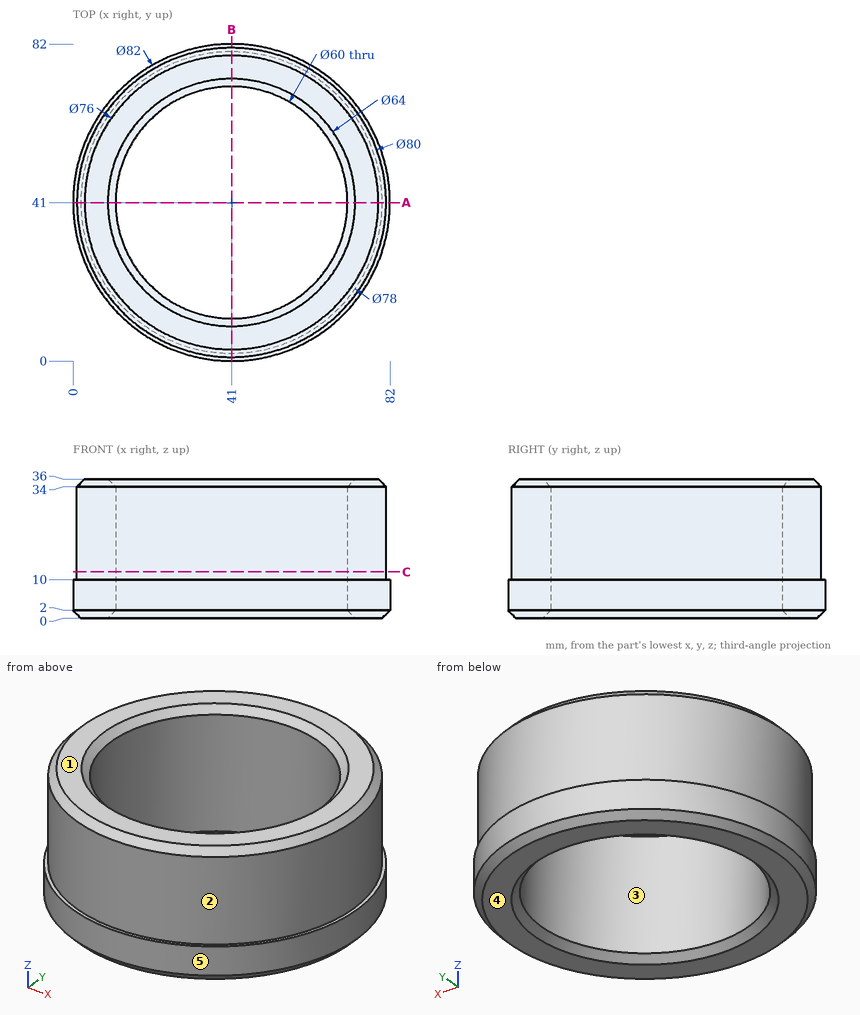
Drawing for the job (mm, zero at the part's lowest x, y, z). A direction names the side the tool comes from. Give positions to 0.01 mm unless a question says otherwise; leave off trailing zeros. Loops run counter-clockwise (first coordinate to the right, second up) from the corner with the lowest first, then second, coordinate; pieces in that order, holes last.
(1) Pin check, flat tips, straight feed: pin 1 (6 mm diameter, centred on y = 57, z = 5, fed in from -X); pin 2 (8 mm diameter, centred on x = 59, z = 20, fed in from +Y); pin 3 (1 mm diameter, centred on y = 60.5, z = 5.5, fed in from +X). Stop position of each tip, or through.
Return value:
pin 1: stops at x = 2.12
pin 2: stops at y = 78.47
pin 3: stops at x = 77.33
(2) 3-axis set-ups, long thin cutter, end or side, ignore diameter. For the marked faces 1 and 2: which of +Z, -Z, +X, -X, +Y, -Y reach the whole face in a straight line?
Return value:
face 1: +Z, +X, -X, +Y, -Y
face 2: +Z
(3) Band-saw the part on A-A (y = 41). Write the cut outline in (x, z).
Return value:
outline: (0, 2) - (2, 0) - (9, 0) - (11, 2) - (11, 34) - (9, 36) - (3, 36) - (1, 34) - (1, 10) - (0, 10) - close; (71, 2) - (73, 0) - (80, 0) - (82, 2) - (82, 10) - (81, 10) - (81, 34) - (79, 36) - (73, 36) - (71, 34) - close
(4) Band-saw the part on C-C (z = 12). Write the cut outline in (x, y), and give its area (3 significant figures).
Return value:
outline: circle Ø80 at (41, 41); hole circle Ø60 at (41, 41)
area: 2,200 mm2
(5) Drill centre lines: line 1 along Y through (x, z) = (41, 15); line 2 along X through (y, z) = (18.5, 34.5); line 3 along X through (y, z) = (38.5, 30). Where is each one in solid material? Low to high.
Return value:
line 1: y = 1 to 11, 71 to 81
line 2: x = 8.53 to 20.41, 61.59 to 73.47
line 3: x = 1.08 to 11.1, 70.9 to 80.92
(6) Pull direction X, two halves, no side cores. Call the marked faces 3, 4 and 5: pulls with the +X half, pulls with the -X half, needs draft (parallel to the pull), parting line crosses it, or undercut.
Return value:
face 3: undercut
face 4: needs draft
face 5: parting line crosses it
